Here's the drawing with two shaded views (mm, measured from the low corner). I have some questions. Give positions to 0.01 mm unless a question says otherwise; leave off trailing zeros. Loops run counter-clockwise (first coordinate to the right, second up) from the corner with the lowest first, then second, coordinate; pieces in that order, holes last. Notation, with made-up numbers: (69.5, 87.25) - (122.5, 87.25) arc R24 ccw to (122.5, 113.25) - close; hole circle Ø2 at (69.25, -18.5). An arc over 180 degrees is marked (long way). Use one line per item in the form item = value.
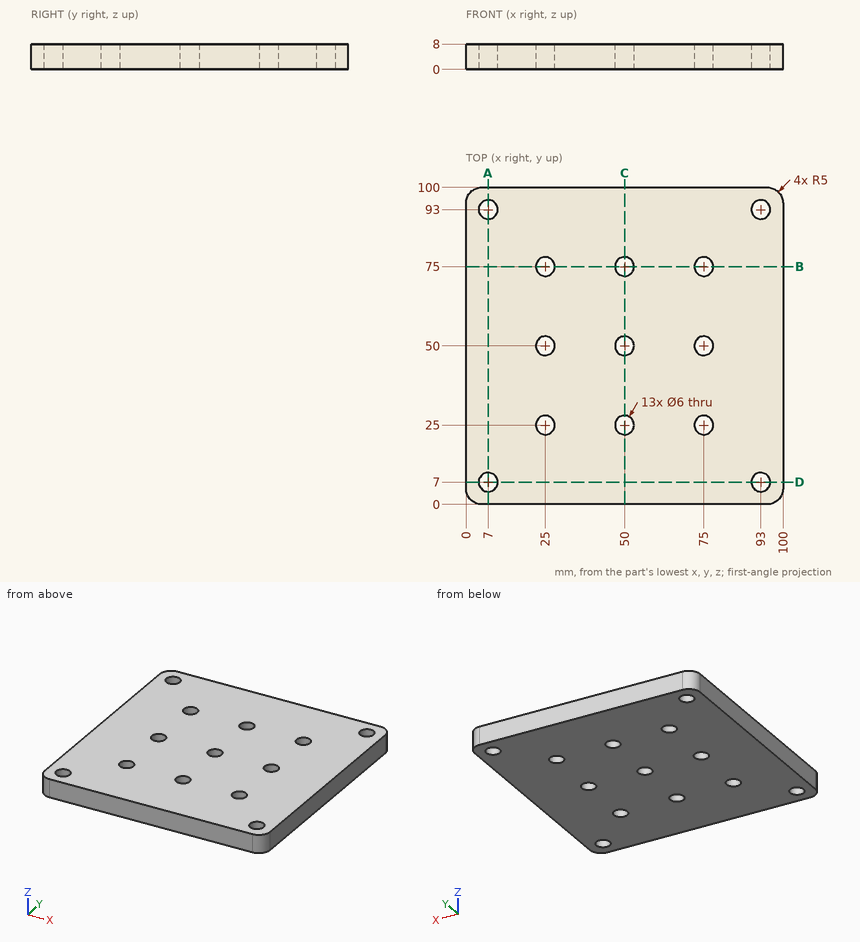
(1) If we section it at B-B (y = 75): List the corners of the cut face in (x, z) for me, plus the area to 3 significant figures.
Geometry says:
outline = (0, 0) - (22, 0) - (22, 8) - (0, 8) - close; (28, 0) - (47, 0) - (47, 8) - (28, 8) - close; (53, 0) - (72, 0) - (72, 8) - (53, 8) - close; (78, 0) - (100, 0) - (100, 8) - (78, 8) - close
area = 656 mm²
(2) For P1, Ø5.5, axis at x = 25, y = 75, coming from the +Z side, with a flat end and sliding along its axis, tell me the tip position at first contact or that it passes through.
Geometry says:
P1 = through
(3) If I drill on probe 1 along Y at (x, z) = (75, 3.5); probe 2 along Y at (x, z) = (22.5, 2); probe 3 along X at (y, z) = (95.5, 2), over which ranges is the centre line in solid material (lowest first)?
Geometry says:
probe_1 = 0 to 22, 28 to 47, 53 to 72, 78 to 100
probe_2 = 0 to 23.34, 26.66 to 48.34, 51.66 to 73.34, 76.66 to 100
probe_3 = 0.03 to 5.34, 8.66 to 91.34, 94.66 to 99.97
(4) If we section it at A-A (x = 7): List the corners of the cut face in (y, z) for me.
Geometry says:
outline = (0, 0) - (4, 0) - (4, 8) - (0, 8) - close; (10, 0) - (90, 0) - (90, 8) - (10, 8) - close; (96, 0) - (100, 0) - (100, 8) - (96, 8) - close
